```python
from build123d import *

# Parameters (mm, degrees)
CUT_EXTRUDE1_REACH = 146.568
SKETCH3_R          = 5
CIRPATTERN1_COUNT  = 6
FILLET1_R          = 10


with BuildPart() as part:
    # Sketch1 → Revolve1 (revolve)
    with BuildSketch(Plane.XY):
        Polygon((0, 25), (0, 100), (20, 100), (20, 50), (50, 50), (50, 25), align=None)
    revolve(axis=Axis((113.213850314, 0, 0), (-1, 0, 0)))

    # Sketch3 → Cut-Extrude1 (cut, up to next)
    with BuildSketch(Plane(origin=(20, 0, 0), x_dir=(0, 0, -1), z_dir=(1, 0, 0)), mode=Mode.PRIVATE) as cut_extrude1_sk1:
        with Locations(Location((0, 75, 0), (0, 0, 90))):
            Circle(SKETCH3_R)
    cut_extrude1_tool1 = extrude(cut_extrude1_sk1.sketch, amount=-CUT_EXTRUDE1_REACH, mode=Mode.PRIVATE) & part.part
    cut_extrude1 = cut_extrude1_tool1.solids().sort_by_distance((20, 75, 0))[0]
    add(cut_extrude1, mode=Mode.SUBTRACT)

    # CirPattern1: Cut-Extrude1 ×6 about axis
    cirpattern1_axis = Axis((0, 0, 0), (1, 0, 0))
    for i in range(1, CIRPATTERN1_COUNT):
        add(cut_extrude1.rotate(cirpattern1_axis, i * 360 / CIRPATTERN1_COUNT), mode=Mode.SUBTRACT)

    # Fillet1
    fillet1_edges = [part.edges().sort_by_distance(p)[0] for p in [
        (50, -50, 0),
    ]]
    fillet(fillet1_edges, radius=FILLET1_R)


solid = part.part
```
Geometry check sheet. Reference: the model listing, model coordinates, mm. A direction names the side the tool comes from. Coordinates: 2 decimals unless noted, no trailing zeros. Order: outer loops, then holes, each group sorted by start corner. A loop starts at its lowest first (then second) coordinate and runs counter-clockwise, first axis right, second up.
Q1. Sectioned sample at B-B on y = 0. Record the cut outline in (x, z).
Reply:
outline: (0, -100) - (20, -100) - (20, -50) - (40, -50) arc R10 ccw to (50, -40) - (50, -25) - (0, -25) - close; (0, 25) - (50, 25) - (50, 40) arc R10 ccw to (40, 50) - (20, 50) - (20, 100) - (0, 100) - close
Q2. Sectioned sample at D-D on x = 31.5. Record the cut outline in (y, z).
Reply:
outline: circle Ø100 at (0, 0); hole circle Ø50 at (0, 0)
Q3. Sectioned sample at C-C on x = 7. Record the cut outline in (y, z).
Reply:
outline: circle Ø200 at (0, 0); hole circle Ø10 at (-75, 0); hole circle Ø10 at (-37.5, -64.95); hole circle Ø10 at (-37.5, 64.95); hole circle Ø50 at (0, 0); hole circle Ø10 at (37.5, -64.95); hole circle Ø10 at (37.5, 64.95); hole circle Ø10 at (75, 0)
Q4. Sectioned sample at A-A on z = 0. Record the cut outline in (x, y).
Reply:
outline: (0, -100) - (20, -100) - (20, -80) - (0, -80) - close; (0, -70) - (20, -70) - (20, -50) - (40, -50) arc R10 ccw to (50, -40) - (50, -25) - (0, -25) - close; (0, 25) - (50, 25) - (50, 40) arc R10 ccw to (40, 50) - (20, 50) - (20, 70) - (0, 70) - close; (0, 80) - (20, 80) - (20, 100) - (0, 100) - close
Q5. Depth check by flat-ended pin: pin 1 Ø1 at (x, z) = (19, -2.5) entering from -Y; pin 2 Ø6 at (y, z) = (16, -47) entering from +X; pin 3 Ø1.5 at (x, y) = (20, 49) entering from -Z. Enter the tip coordinate at first touch or a pass-through.
Reply:
pin 1: stops at y = -99.98
pin 2: stops at x = 47.47
pin 3: stops at z = -87.59
Q6. Draft check along Z on faces 1 (the face through (10.14, 95.38, -30.04)), 2 (the face through (10.14, 79.619, -1.915)), 3 (the face through (20, -46, 21)). Enter one of: released by +Z, released by -Z, zero draft, split by the parting line, or undercut.
Reply:
face 1: split by the parting line
face 2: undercut
face 3: zero draft
Q7. Thickness scan on probe 1 along Z at (x, y) = (11, 0); probe 2 along Y at (x, z) = (3.5, -61.5); probe 3 along Z at (x, y) = (13.5, 37.5). Record the ranges inside material, lowest first.
Reply:
probe 1: z = -100 to -25, 25 to 100
probe 2: y = -78.85 to -41.12, -33.88 to 33.88, 41.12 to 78.85
probe 3: z = -92.7 to -69.95, -59.95 to 59.95, 69.95 to 92.7
Q8. Tool access check on faces 4 (the face through (10.14, -38.15, 69.91)), 5 (the face through (30.14, 47.69, -15.02)). Record the directions out of +Z, -Z, +X, -X, +Y, -Y that give a thin tool (end or side, any length) a straight path to the whole face; none if there is none.
Reply:
face 4: +X, -X
face 5: +X
